Could you check a few things on this model? Use its own coordinates, in mm. Face numbers are marked on the shaded views. A direction names the side the tool comes from. Coordinates: 2 decimals unless noted, no trailing zeros. Order: outer loops, then holes, each group sorted by start corner. A loop starts at its lowest first (then second) coordinate and runs counter-clockwise, first axis right, second up. Notation, with made-up numbers: (32.5, 17.25) - (38.5, 17.25) arc R31 cw to (38.5, 52.25) - close; hole circle Ø4 at (53, 2.25). An arc over 180 degrees is marked (long way). Answer as CSV lines item,"result". Start each with the question number.
1. I need wall thicknesses on probe 1 along Z at (x, y) = (39.5, 23.5); probe 2 along Z at (x, y) = (67.5, 24); probe 3 along X at (y, z) = (27, 13). Which ranges of each line are inside material? Lowest first, please.
2. For pin 1 (0.9 mm diameter, centred on x = 73.5, z = 29.5, fed in from -Y); pin 2 (4 mm diameter, centred on y = -13.5, z = 28, fed in from -X); pin 3 (2.5 mm diameter, centred on x = 80, y = -29.5, fed in from -Z), each with a flat end and sliding along its axis, tell me the tip position at first contact or that it passes through.
3. Thinking about a two-plate mould opening in Y: for the marked faces 1, 2 and 3, which applies, released by +Y, released by -Y, zero draft, split by the parting line, or undercut?
4. I want a section at D-D, the plane x = -13.5. List the corners of the cut face in (y, z) for me, and give its area (3 significant figures).
5. I want a section at A-A, the plane y = 0. List the corners of the cut face in (x, z) for me.
6. I want a section at C-C, the plane z = -12.5. List the corners of the cut face in (x, y) for me, and give its area (3 significant figures).
7. For the marked faces 4, 5, 6, 7 and 8, which set-ups out of +Z, -Z, +X, -X, +Y, -Y let a thin tool reach every point of the face, with its end or its side?
from build123d import *

# Parameters (mm, degrees)
BOSS_EXTRUDE1_DEPTH = 82
CIRPATTERN1_COUNT   = 8
SKETCH3_R           = 25
BOSS_EXTRUDE2_DEPTH = 30


with BuildPart() as part:
    # Sketch1 → Revolve1 (revolve)
    with BuildSketch(Plane(origin=(0, 0, 0), x_dir=(1, 0, 0), z_dir=(0, 1, 0))):
        Polygon((0, 0), (0, 31), (11, 31), (11, 36), (31, 36), (31, 28), (113, 28), (113, 0), align=None)
    revolve(axis=Axis((113, 0, 0), (-1, 0, 0)))

    # Sketch2 → Boss-Extrude1 (add)
    with BuildSketch(Plane(origin=(113, 0, 0), x_dir=(0, 0, -1), z_dir=(1, 0, 0))):
        with BuildLine():
            Line((-5, 30.594117082), (-5, 27.549954628))
            ThreePointArc((-5, 27.549954628), (0, 28), (5, 27.549954628))
            Line((5, 27.549954628), (5, 30.594117082))
            ThreePointArc((5, 30.594117082), (0, 31), (-5, 30.594117082))
        make_face()
    boss_extrude1 = extrude(amount=-BOSS_EXTRUDE1_DEPTH)

    # CirPattern1: Boss-Extrude1 ×8 about axis
    cirpattern1_axis = Axis((0, 0, 0), (1, 0, 0))
    for i in range(1, CIRPATTERN1_COUNT):
        add(boss_extrude1.rotate(cirpattern1_axis, i * 360 / CIRPATTERN1_COUNT))

    # Sketch3 → Boss-Extrude2 (add)
    with BuildSketch(Plane.ZY):
        Circle(SKETCH3_R)
    extrude(amount=BOSS_EXTRUDE2_DEPTH)


solid = part.part
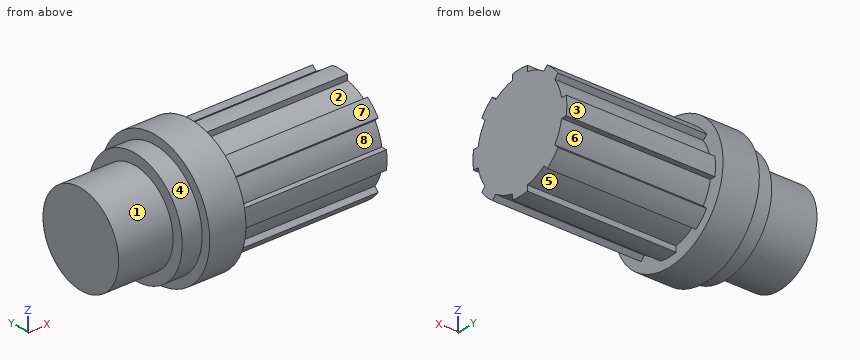
Solved:
1,probe 1,"z = -20.22 to -16.43, -15.22 to 15.22, 16.43 to 20.22"
1,probe 2,"z = -19.62 to -16.93, -14.42 to 14.42, 16.93 to 19.62"
1,probe 3,"x = 0 to 31"
2,pin 1,"stops at y = -5"
2,pin 2,"stops at x = 0"
2,pin 3,"stops at z = -5"
3,face 1,"split by the parting line"
3,face 2,"undercut"
3,face 3,"released by +Y"
4,outline,"circle Ø50 at (0, 0)"
4,area,"1,960 mm2"
5,outline,"(-30, -25) - (0, -25) - (0, -31) - (11, -31) - (11, -36) - (31, -36) - (31, -31) - (113, -31) - (113, 31) - (31, 31) - (31, 36) - (11, 36) - (11, 31) - (0, 31) - (0, 25) - (-30, 25) - close"
6,outline,"(-30, -21.65) - (0, -21.65) - (0, -28.37) - (11, -28.37) - (11, -33.76) - (31, -33.76) - (31, -25.05) - (113, -25.05) - (113, 25.05) - (31, 25.05) - (31, 33.76) - (11, 33.76) - (11, 28.37) - (0, 28.37) - (0, 21.65) - (-30, 21.65) - close"
6,area,"7,380 mm2"
7,face 4,"-X"
7,face 5,"-Z, +X"
7,face 6,"+X, +Y"
7,face 7,"+Z, +X, -Y"
7,face 8,"+X, -Y"
